from build123d import *

# Parameters (mm, degrees)
SKETCH_1_W          = 110
SKETCH_1_H          = 100
EXTRUDE_1_DEPTH     = 5
CUT_EXTRUDE_1_DEPTH = 5
SKETCH_3_W          = 5
SKETCH_3_H          = 100
EXTRUDE_2_DEPTH     = 50
SKETCH_4_W          = 5
SKETCH_4_H          = 100
EXTRUDE_3_DEPTH     = 50
SKETCH_5_W          = 5
SKETCH_5_H          = 100
CUT_EXTRUDE_2_DEPTH = 50
SKETCH_7_W          = 5
SKETCH_7_H          = 100
CUT_EXTRUDE_3_DEPTH = 50


with BuildPart() as part:
    # Sketch 1 → Extrude 1 (new body)
    with BuildSketch(Plane.XY):
        with Locations((55, 50)):
            Rectangle(SKETCH_1_W, SKETCH_1_H)
    extrude(amount=EXTRUDE_1_DEPTH)

    # Sketch 2 → Cut-Extrude 1 (cut)
    with BuildSketch(Plane.XY.offset(5)):
        with BuildLine():
            Line((55, 50), (79.048052385, 71.861865805))
            ThreePointArc((79.048052385, 71.861865805), (68.147991507, 79.72171461), (55, 82.5))
            Line((55, 82.5), (55, 50))
        make_face()
        with BuildLine():
            Line((30.951947615, 28.138134195), (55, 50))
            Line((55, 50), (55, 82.5))
            ThreePointArc((55, 82.5), (25.27828539, 63.147991507), (30.951947615, 28.138134195))
        make_face()
        with BuildLine():
            ThreePointArc((87.5, 50), (85.313459903, 61.719391995), (79.048052385, 71.861865805))
            Line((79.048052385, 71.861865805), (55, 50))
            Line((55, 50), (30.951947615, 28.138134195))
            ThreePointArc((30.951947615, 28.138134195), (66.719391995, 19.686540097), (87.5, 50))
        make_face()
    extrude(amount=-CUT_EXTRUDE_1_DEPTH, mode=Mode.SUBTRACT)

    # Sketch 3 → Extrude 2 (add)
    with BuildSketch(Plane(origin=(110, 0, 0), x_dir=(0, 0, -1), z_dir=(1, 0, 0))):
        with Locations((-2.5, 50)):
            Rectangle(SKETCH_3_W, SKETCH_3_H)
    extrude(amount=EXTRUDE_2_DEPTH)

    # Sketch 4 → Extrude 3 (add)
    with BuildSketch(Plane.ZY):
        with Locations((2.5, 50)):
            Rectangle(SKETCH_4_W, SKETCH_4_H)
    extrude(amount=EXTRUDE_3_DEPTH)

    # Sketch 5 → Cut-Extrude 2 (cut)
    with BuildSketch(Plane(origin=(160, 0, 0), x_dir=(0, 0, -1), z_dir=(1, 0, 0))):
        with Locations((-2.5, 50)):
            Rectangle(SKETCH_5_W, SKETCH_5_H)
    extrude(amount=-CUT_EXTRUDE_2_DEPTH, mode=Mode.SUBTRACT)

    # Sketch 7 → Cut-Extrude 3 (cut)
    with BuildSketch(Plane.ZY.offset(50)):
        with Locations((2.5, 50)):
            Rectangle(SKETCH_7_W, SKETCH_7_H)
    extrude(amount=-CUT_EXTRUDE_3_DEPTH, mode=Mode.SUBTRACT)


solid = part.part
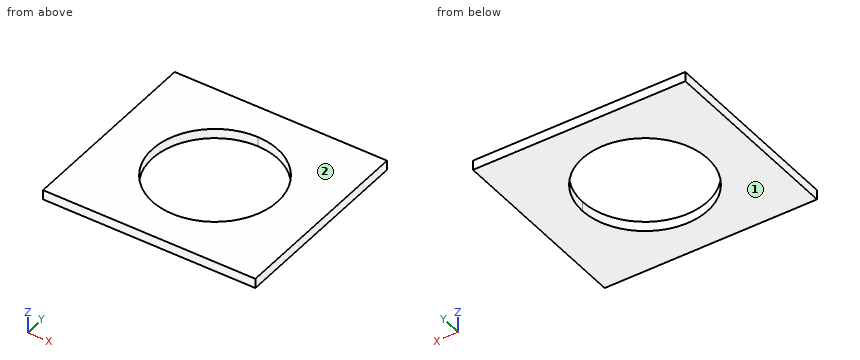
Read the model definition and answer for the solid it produces. Units are mm, in the model's axes. Face numbers are marked on the shaded views. Give positions to 0.01 mm unless a question says otherwise; leave off trailing zeros. Write each loop counter-clockwise with the first axis right and the second up, starting at its lowest first coordinate (ties: lowest second). Pieces come first, ordered by that corner, then holes. Notation, with made-up numbers: (76, 82.25) - (105, 82.25) arc R29 ccw to (105, 102.25) - close; hole circle Ø1 at (-13, -17). An arc over 180 degrees is marked (long way). Use CSV: the item, a comma, the result in double quotes. Start each with the question number.
Item 1: The part is cut by section B-B, the plane y = 42. Give the vertices of the cut face in (x, z), and give its area (3 significant figures).
Item 2: The mould has two halves that part along Z. Classify the marked faces 1 and 2: pulls with the +Z half, pulls with the -Z half, needs draft (parallel to the pull), parting line crosses it, or undercut.
Item 3: The part is cut by section C-C, the plane x = 84.5. Give the vertices of the cut face in (y, z), and give its area (3 significant figures).
Item 4: The part is cut by section A-A, the plane z = 3.05. Give the vertices of the cut face in (x, y).
Item 5: Consider line 1 (Y direction, x = 68, z = 1.05); line 2 (X direction, y = 55, z = 3); line 3 (X direction, y = 48.5, z = 0.5). Determine where each line is inside the solid, lowest interval first.
Taken from the geometry:
1,outline,"(0, 0) - (23.5, 0) - (23.5, 5) - (0, 5) - close; (86.5, 0) - (110, 0) - (110, 5) - (86.5, 5) - close"
1,area,"235 mm2"
2,face 1,"pulls with the -Z half"
2,face 2,"pulls with the +Z half"
3,outline,"(0, 0) - (36.36, 0) - (36.36, 5) - (0, 5) - close; (63.64, 0) - (100, 0) - (100, 5) - (63.64, 5) - close"
3,area,"364 mm2"
4,outline,"(0, 0) - (110, 0) - (110, 100) - (0, 100) - close; hole circle Ø65 at (55, 50)"
5,line 1,"0 to 20.21, 79.79 to 100"
5,line 2,"0 to 22.89, 87.11 to 110"
5,line 3,"0 to 22.53, 87.47 to 110"
